Build history of the part. All positions in model axes, mm. Give positions to 0.01 mm unless a question says otherwise; leave off trailing zeros. Loops run counter-clockwise (first coordinate to the right, second up) from the corner with the lowest first, then second, coordinate; pieces in that order, holes last. Notation, with made-up numbers: (24, 57.25) -> (38, 57.25) arc R33 ccw to (38, 95.25) -> close; hole circle Ø7 at (9.25, 3.5). An arc over 180 degrees is marked (long way). Answer as a JSON object with one key per item and string values. Group by question number.
from build123d import *

# Parameters (mm, degrees)
SKETCH_1_W          = 20
SKETCH_1_H          = 20
EXTRUDE_1_DEPTH     = 350
SKETCH_2_R          = 3.5
CUT_EXTRUDE_1_DEPTH = 700


with BuildPart() as part:
    # 草图1 → 凸台-拉伸1 (new, symmetric)
    with BuildSketch(Plane(origin=(0, 0, 0), x_dir=(0, 0, -1), z_dir=(1, 0, 0))):
        Rectangle(SKETCH_1_W, SKETCH_1_H)
    extrude(amount=EXTRUDE_1_DEPTH, both=True)

    # 草图2 → 切除-拉伸1 (cut)
    with BuildSketch(Plane.XY.offset(10)):
        with Locations((-45, 0)):
            Circle(SKETCH_2_R)
        with Locations((45, 0)):
            Circle(SKETCH_2_R)
    extrude(amount=-CUT_EXTRUDE_1_DEPTH, mode=Mode.SUBTRACT)


solid = part.part
(1) Probe line 1 along Y through (x, z) = (-45, 3.25); line 2 along X through (y, z) = (-2, -2.25); line 3 along X through (y, z) = (1.75, -6.5). List the from-to ranges inside material, lowest first. Write a range as [from, to].
(2) Pin check, flat tip, straight feed: pin 1 (6.5 mm diameter, centred on x = 45, y = 0, fed in from +Z). Stop position of the tip, or through.
(3) Saw through at A-A on y = 0. List the corners of the cut face in (x, z).
Calculated:
{
 "1": {"line 1": "y = [-10, -3.5], [3.5, 10]", "line 2": "x = [-350, -47.87], [-42.13, 42.13], [47.87, 350]", "line 3": "x = [-350, -48.03], [-41.97, 41.97], [48.03, 350]"},
 "2": {"pin 1": "passes through"},
 "3": {"outline": "(-350, -10) -> (-48.5, -10) -> (-48.5, 10) -> (-350, 10) -> close; (-41.5, -10) -> (41.5, -10) -> (41.5, 10) -> (-41.5, 10) -> close; (48.5, -10) -> (350, -10) -> (350, 10) -> (48.5, 10) -> close"}
}
